Work out the finished part from the listing and answer in its coordinate system (mm). Face numbers are marked on the shaded views. A direction names the side the tool comes from. Give positions to 0.01 mm unless a question says otherwise; leave off trailing zeros. Loops run counter-clockwise (first coordinate to the right, second up) from the corner with the lowest first, then second, coordinate; pieces in that order, holes last. Notation, with made-up numbers: M 25,40.5 L 57,40.5 A33 cw 57,73.5 Z; hole C 26,-16.5 d4. An arc over 180 degrees is marked long. Use a Markdown table: item, result.
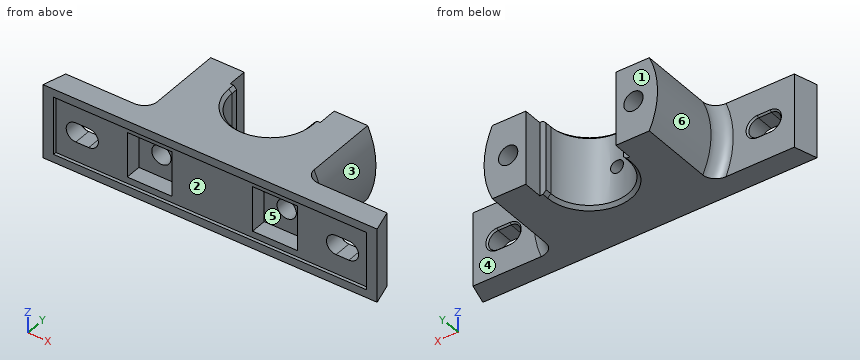
```python
from build123d import *

# Parameters (mm, degrees)
BASE_PLATE_SKETCH_W             = 208
BASE_PLATE_SKETCH_H             = 46
BASE_PLATE_208X46X14_DEPTH      = 14
BASE_END_BEVEL_SKETCH_OUTSIDE_W = 252.698
BASE_END_BEVEL_SKETCH_OUTSIDE_H = 58.698
BASE_END_BEVELS_DEPTH           = 115.577484699
BEARING_PEDESTAL_DEPTH          = 46
UNDERSIDE_RELIEF_SKETCH_W       = 195
UNDERSIDE_RELIEF_SKETCH_H       = 36
UNDERSIDE_RELIEF_2MM_DEPTH      = 2
BEARING_BORE_SKETCH_W           = 28
BEARING_BORE_SKETCH_H           = 28
BEARING_BORE_CUT_DEPTH          = 10
MOUNTING_SLOTS_2X8_DEPTH        = 127.368508735
CAP_BOLT_HOLES_2X_12_D          = 12
PEDESTAL_CHAMFER_2MM_SIZE       = 2
SLOT_EDGE_CHAMFER_1MM_SIZE      = 1
DRILLED_HOLE_8_D                = 8
DRILLED_HOLE_8_DEPTH            = 36
PEDESTAL_PROFILE_CUT_DEPTH      = 54
PEDESTAL_BASE_FILLET_R8_R       = 8


with BuildPart() as part:
    # Base Plate Sketch → Base Plate 208x46x14 (new body)
    with BuildSketch(Plane(origin=(0, 0, 0), x_dir=(1, 0, 0), z_dir=(0, 1, 0))):
        Rectangle(BASE_PLATE_SKETCH_W, BASE_PLATE_SKETCH_H)
    extrude(amount=BASE_PLATE_208X46X14_DEPTH)

    # Base End Bevel Sketch outside → Base End Bevels (cut, through all)
    with BuildSketch(Plane.XY.offset(23)):
        with Locations((0, 7)):
            Rectangle(BASE_END_BEVEL_SKETCH_OUTSIDE_W, BASE_END_BEVEL_SKETCH_OUTSIDE_H)
        Polygon((-104, 0), (-99.985564599, 14), (99.985564599, 14), (104, 0), align=None, mode=Mode.SUBTRACT)
    extrude(amount=-BASE_END_BEVELS_DEPTH, mode=Mode.SUBTRACT)

    # Pedestal Sketch → Bearing Pedestal (add, through all)
    with BuildSketch(Plane.XY.offset(23)):
        with BuildLine():
            Line((-56, 14), (56, 14))
            Line((56, 14), (56, 68))
            Line((56, 68), (28, 68))
            Line((28, 68), (28, 56))
            Line((28, 56), (24, 56))
            Line((24, 56), (24, 52))
            ThreePointArc((24, 52), (0, 28), (-24, 52))
            Line((-24, 52), (-24, 56))
            Line((-24, 56), (-28, 56))
            Line((-28, 56), (-28, 68))
            Line((-28, 68), (-56, 68))
            Line((-56, 68), (-56, 14))
        make_face()
    extrude(amount=-BEARING_PEDESTAL_DEPTH)

    # Underside Relief Sketch → Underside Relief 2mm (cut)
    with BuildSketch(Plane.XZ):
        Rectangle(UNDERSIDE_RELIEF_SKETCH_W, UNDERSIDE_RELIEF_SKETCH_H)
    extrude(amount=-UNDERSIDE_RELIEF_2MM_DEPTH, mode=Mode.SUBTRACT)

    # Bearing Bore Sketch → Bearing Bore Cut (cut)
    with BuildSketch(Plane.XZ.offset(-2)):
        with Locations((39, 0)):
            Rectangle(BEARING_BORE_SKETCH_W, BEARING_BORE_SKETCH_H)
        with Locations((-39, 0)):
            Rectangle(BEARING_BORE_SKETCH_W, BEARING_BORE_SKETCH_H)
    extrude(amount=-BEARING_BORE_CUT_DEPTH, mode=Mode.SUBTRACT)

    # Mounting Slots Sketch → Mounting Slots 2x8 (cut, through all)
    with BuildSketch(Plane(origin=(0, 0, 0), x_dir=(1, 0, 0), z_dir=(0, 1, 0))):
        with BuildLine():
            Line((77, 6), (85, 6))
            ThreePointArc((85, 6), (91, 0), (85, -6))
            Line((85, -6), (77, -6))
            ThreePointArc((77, -6), (71, 0), (77, 6))
        make_face()
        with BuildLine():
            Line((-77, 6), (-85, 6))
            ThreePointArc((-85, 6), (-91, 0), (-85, -6))
            Line((-85, -6), (-77, -6))
            ThreePointArc((-77, -6), (-71, 0), (-77, 6))
        make_face()
    extrude(amount=MOUNTING_SLOTS_2X8_DEPTH, mode=Mode.SUBTRACT)

    # Cap Bolt Holes 2xØ12 (through all)
    with Locations(Plane(origin=(0, 12, 0), x_dir=(-1, 0, 0), z_dir=(0, -1, 0))):
        with Locations((-39, 0), (39, 0)):
            Hole(CAP_BOLT_HOLES_2X_12_D / 2)

    # Pedestal Chamfer 2mm
    pedestal_chamfer_2mm_edges = [part.edges().sort_by_distance(p)[0] for p in [
        (-24, 54, -23),
        (0, 28, -23),
        (24, 54, -23),
        (24, 54, 23),
        (0, 28, 23),
        (-24, 54, 23),
    ]]
    chamfer(pedestal_chamfer_2mm_edges, length=PEDESTAL_CHAMFER_2MM_SIZE)

    # Slot Edge Chamfer 1mm
    slot_edge_chamfer_1mm_edges = [part.edges().sort_by_distance(p)[0] for p in [
        (71, 14, 0),
        (81, 14, 6),
        (91, 14, 0),
        (81, 14, -6),
        (-71, 14, 0),
        (-81, 14, -6),
        (-91, 14, 0),
        (-81, 14, 6),
    ]]
    chamfer(slot_edge_chamfer_1mm_edges, length=SLOT_EDGE_CHAMFER_1MM_SIZE)

    # Drilled Hole Ø8
    with Locations(Plane(origin=(0, 56, 0), x_dir=(1, 0, 0), z_dir=(0, 1, 0))):
        with Locations((0, 0)):
            Hole(DRILLED_HOLE_8_D / 2, depth=DRILLED_HOLE_8_DEPTH)

    # Pedestal Profile Sketch → Pedestal Profile Cut (cut)
    with BuildSketch(Plane(origin=(0, 68, 0), x_dir=(1, 0, 0), z_dir=(0, 1, 0))):
        with BuildLine():
            Line((-56, -23), (-48.856934001, -23))
            ThreePointArc((-48.856934001, -23), (-54, 0), (-48.856934001, 23))
            Line((-48.856934001, 23), (-56, 23))
            Line((-56, 23), (-56, -23))
        make_face()
        with BuildLine():
            Line((48.856934001, -23), (56, -23))
            Line((56, -23), (56, 23))
            Line((56, 23), (48.856934001, 23))
            ThreePointArc((48.856934001, 23), (54, 0), (48.856934001, -23))
        make_face()
    extrude(amount=-PEDESTAL_PROFILE_CUT_DEPTH, mode=Mode.SUBTRACT)

    # Pedestal Base Fillet R8
    pedestal_base_fillet_r8_edges = [part.edges().sort_by_distance(p)[0] for p in [
        (-54, 14, 0),
        (54, 14, 0),
    ]]
    fillet(pedestal_base_fillet_r8_edges, radius=PEDESTAL_BASE_FILLET_R8_R)


solid = part.part
```
(1) A cutting plane is placed at C-C (z = 0). Count the separate pieces of the cut face and the enclosed holes in it, and give its area (3 significant figures).
Entries:
| item | result |
|---|---|
| separate pieces | 5 |
| enclosed holes | 0 |
| area | 4,110 mm² |
(2) The mould has two halves that part along X. Classify the marked faces 3, 4, 5 and 6: released by +X, released by -X, zero draft, split by the parting line, or undercut.
Entries:
| item | result |
|---|---|
| face 3 | released by +X |
| face 4 | zero draft |
| face 5 | undercut |
| face 6 | released by -X |
(3) A cutting plane is placed at A-A (y = 63). Write down the section's boundary in (x, z), and give its area (3 significant figures).
Entries:
| item | result |
|---|---|
| outline | M -48.86,-23 L -28,-23 L -28,23 L -48.86,23 A54 ccw Z; M 28,-23 L 48.86,-23 A54 ccw 48.86,23 L 28,23 Z; hole C -39,0 d12; hole C 39,0 d12 |
| area | 2,010 mm² |
(4) Consider probe 1 along Z at (x, y) = (-39, 47); probe 2 along X at (y, z) = (22.5, -2); probe 3 along Y at (x, z) = (85.5, 10). Determine where each line is inside the solid, lowest interval first. Write a range as [from, to].
Entries:
| item | result |
|---|---|
| probe 1 | z = [-23, -6], [6, 23] |
| probe 2 | x = [-53.96, -44.66], [-33.34, -3.46], [3.46, 33.34], [44.66, 53.96] |
| probe 3 | y = [2, 14] |
(5) A cutting plane is placed at B-B (x = -39). Write down the section's boundary in (y, z), and give its area (3 significant figures).
Entries:
| item | result |
|---|---|
| outline | M 0,-23 L 68,-23 L 68,-6 L 12,-6 L 12,-14 L 2,-14 L 2,-18 L 0,-18 Z; M 0,18 L 2,18 L 2,14 L 12,14 L 12,6 L 68,6 L 68,23 L 0,23 Z |
| area | 2,100 mm² |
(6) Given P1, Ø12, axis at x = -22.5, z = -3, coming from the +Y side; P2, Ø6, axis at y = 52.5, z = -12, coming from the -X side; P3, Ø12, axis at y = 23.5, z = 12, coming from the +X side; P4, Ø11, axis at y = 7.5, z = -6, coming from the +X side, each flat-ended and moving along its own axis, determine where each tip first touches the part or whether it passes through.
Entries:
| item | result |
|---|---|
| P1 | stops at y = 68 |
| P2 | stops at x = -53.24 |
| P3 | stops at x = 54.26 |
| P4 | stops at x = 103.43 |
(7) A cutting plane is placed at D-D (x = 0). Write down the section's boundary in (y, z), and give its area (3 significant figures).
Entries:
| item | result |
|---|---|
| outline | M 0,-23 L 26,-23 L 28,-21 L 28,-4 L 20,-4 L 20,4 L 28,4 L 28,21 L 26,23 L 0,23 L 0,18 L 2,18 L 2,-18 L 0,-18 Z |
| area | 1,150 mm² |
(8) Which of the six approach directions +Z, -Z, +X, -X, +Y, -Y give full straight-line access (tool end or side, diameter ignored) to the marked faces 1 and 2?
Entries:
| item | result |
|---|---|
| face 1 | +Z, -Z, +X, -X, +Y |
| face 2 | -Y |
